from build123d import *

# Parameters (mm, degrees)
SKETCH_1_W                = 95
SKETCH_1_H                = 155
EXTRUDE_1_DEPTH           = 12
SKETCH_9_W                = 15.5
SKETCH_9_H                = 143
CUT_EXTRUDE_4_DEPTH       = 183.1922062
HOLE_WIZARD_6_5_6_5_1_D   = 6.5
SKETCH_12_R               = 17.5
CUT_EXTRUDE_5_DEPTH       = 183.1922062
FILLET_1_R                = 10
HOLE_WIZARD_5_0_5_1_D     = 5
HOLE_WIZARD_5_0_5_1_DEPTH = 10
HOLE_WIZARD_5_0_5_1_TIP   = 1.502151548
FILLET_2_R                = 2
HOLE_WIZARD_M6_2_D        = 5
MM_1_D                    = 9


with BuildPart() as part:
    # 草图1 → 凸台-拉伸1 (new body)
    with BuildSketch(Plane(origin=(0, 0, 0), x_dir=(1, 0, 0), z_dir=(0, 1, 0))):
        with Locations((47.5, -77.5)):
            Rectangle(SKETCH_1_W, SKETCH_1_H)
    extrude(amount=EXTRUDE_1_DEPTH)

    # 草图9 → 切除-拉伸4 (cut, through all)
    with BuildSketch(Plane(origin=(0, 12, 0), x_dir=(1, 0, 0), z_dir=(0, 1, 0))):
        with Locations((7.75, -83.5)):
            Rectangle(SKETCH_9_W, SKETCH_9_H)
        with Locations((87.25, -83.5)):
            Rectangle(SKETCH_9_W, SKETCH_9_H)
    extrude(amount=-CUT_EXTRUDE_4_DEPTH, mode=Mode.SUBTRACT)

    # Ø6.5 (6.5) 直径孔1 (through all)
    with Locations(Plane.XY.offset(12)):
        with Locations((6, 6), (89, 6)):
            Hole(HOLE_WIZARD_6_5_6_5_1_D / 2)

    # 草图12 → 切除-拉伸5 (cut, through all)
    with BuildSketch(Plane(origin=(0, 12, 0), x_dir=(1, 0, 0), z_dir=(0, 1, 0))):
        with Locations(Location((47.5, -123, 0), (0, 0, 270))):
            Circle(SKETCH_12_R)
    extrude(amount=-CUT_EXTRUDE_5_DEPTH, mode=Mode.SUBTRACT)

    # 圆角1
    fillet_1_edges = [part.edges().sort_by_distance(p)[0] for p in [
        (15.5, 6, 155),
        (79.5, 6, 155),
    ]]
    fillet(fillet_1_edges, radius=FILLET_1_R)

    # Ø5.0 (5) 直径孔1
    with Locations(Plane(origin=(0, 0, 0), x_dir=(-1, 0, 0), z_dir=(0, 0, -1))):
        with Locations((-67.5, 6), (-27.5, 6)):
            Hole(HOLE_WIZARD_5_0_5_1_D / 2, depth=HOLE_WIZARD_5_0_5_1_DEPTH)
            with Locations((0, 0, -(HOLE_WIZARD_5_0_5_1_DEPTH + HOLE_WIZARD_5_0_5_1_TIP / 2))):  # 118° drill point
                Cone(0, HOLE_WIZARD_5_0_5_1_D / 2, HOLE_WIZARD_5_0_5_1_TIP, mode=Mode.SUBTRACT)

    # 圆角2
    fillet_2_edges = [part.edges().sort_by_distance(p)[0] for p in [
        (15.5, 6, 12),
        (79.5, 6, 12),
    ]]
    fillet(fillet_2_edges, radius=FILLET_2_R)

    # M6 螺纹孔2 (through all)
    with Locations(Plane(origin=(0, 0, 0), x_dir=(-1, 0, 0), z_dir=(0, -1, 0))):
        with Locations((-68.5, -44.5), (-26.5, -44.5)):
            Hole(HOLE_WIZARD_M6_2_D / 2)

    # 大小mm 暗销孔1 (through all)
    with Locations(Plane(origin=(0, 0, 0), x_dir=(-1, 0, 0), z_dir=(0, -1, 0))):
        with Locations((-72.5, -98), (-72.5, -148), (-22.5, -148), (-22.5, -98)):
            Hole(MM_1_D / 2)


solid = part.part
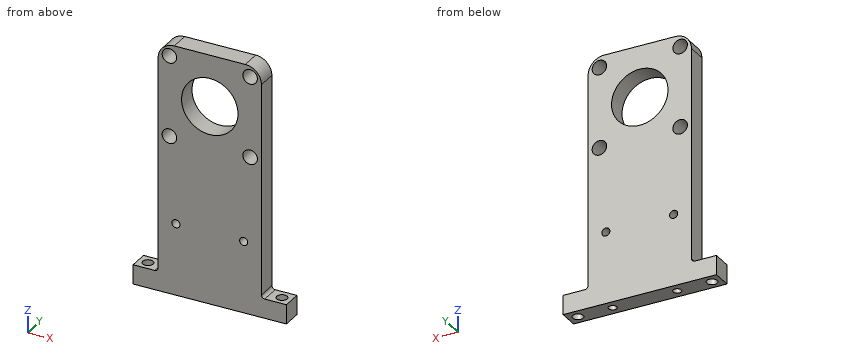
CAD build for the part. Positions are in the model's coordinates, mm. Round coordinates to 2 decimals unless told otherwise and drop trailing zeros. Write each loop counter-clockwise with the first axis right and the second up, starting at its lowest first coordinate (ties: lowest second). Pieces come first, ordered by that corner, then holes. Notation, with made-up numbers: M -30,-25 L 6,-25 A31 ccw 6,6 Z; hole C -13,58.25 d6. An arc over 180 degrees is marked long. Use a Markdown table: item, result. Add a question column.
1. Slice it at A-A on x = 58. Give the cut face in (y, z), then the cut area to 3 significant figures.
2. Flat gauge pins, fed straight in: P1, Ø3.5, axis at y = 5, z = 93.5, coming from the -X side; P2, Ø6, axis at y = 3.5, z = 40.5, coming from the +X side. Where does each tip first touch, or does it go through?
3. Slice it at C-C on z = 44.5. Give the cut face in (x, y).
4. Slice it at D-D on x = 22.5. Give the cut face in (y, z), then the cut area to 3 significant figures.
5. Slice it at B-B on z = 123. Give the cut face in (x, y), then the cut area to 3 significant figures.
6. Drill centre lines: probe 1 along X at (y, z) = (7.75, 44.5); probe 2 along Y at (x, z) = (6, 6); probe 3 along X at (y, z) = (11.25, 94.5). Where is each one in solid material? Low to high.
Reply:
| question | item | result |
|---|---|---|
| 1 | outline | M 0,0 L 12,0 L 12,109 L 0,109 Z; M 0,137 L 12,137 L 12,155 L 0,155 Z |
| 1 | area | 1,520 mm^2 |
| 2 | P1 | stops at x = 15.5 |
| 2 | P2 | stops at x = 79.5 |
| 3 | outline | M 15.5,0 L 24,0 L 24,12 L 15.5,12 Z; M 29,0 L 66,0 L 66,12 L 29,12 Z; M 71,0 L 79.5,0 L 79.5,12 L 71,12 Z |
| 4 | outline | M 0,0 L 12,0 L 12,93.5 L 0,93.5 Z; M 0,102.5 L 12,102.5 L 12,143.5 L 0,143.5 Z; M 0,152.5 L 12,152.5 L 12,154.54 L 0,154.54 Z |
| 4 | area | 1,640 mm^2 |
| 5 | outline | M 15.5,0 L 30,0 L 30,12 L 15.5,12 Z; M 65,0 L 79.5,0 L 79.5,12 L 65,12 Z |
| 5 | area | 348 mm^2 |
| 6 | probe 1 | x = 15.5 to 24, 29 to 66, 71 to 79.5 |
| 6 | probe 2 | y = 0 to 2.75, 9.25 to 12 |
| 6 | probe 3 | x = 15.5 to 19.67, 25.33 to 69.67, 75.33 to 79.5 |
